The listing builds one solid part. Answer for the finished solid, in the listing's coordinates (mm). A direction names the side the tool comes from. Coordinates: 2 decimals unless noted, no trailing zeros. Order: outer loops, then holes, each group sorted by start corner. A loop starts at its lowest first (then second) coordinate and runs counter-clockwise, first axis right, second up.
from build123d import *

# Parameters (mm, degrees)
BOSS_EXTRUDE1_DEPTH = 30
SKETCH2_W           = 45.814700403
SKETCH2_H           = 10
CUT_EXTRUDE1_DEPTH  = 80
CUT_EXTRUDE2_DEPTH  = 10


with BuildPart() as part:
    # Sketch1 → Boss-Extrude1 (new body)
    with BuildSketch(Plane.XY.offset(3001.335718486)):
        with BuildLine():
            Line((917.934929034, 337.734430273), (888.537204265, 331.753311783))
            ThreePointArc((888.537204265, 331.753311783), (884.042481487, 330.053316774), (880.315998683, 327.019203759))
            Line((880.315998683, 327.019203759), (659.406795905, 282.074088861))
            ThreePointArc((659.406795905, 282.074088861), (654.791020678, 283.41092652), (649.989366626, 283.21952579))
            Line((649.989366626, 283.21952579), (620.591641856, 277.2384073))
            ThreePointArc((620.591641856, 277.2384073), (608.883338717, 259.54898567), (626.572760347, 247.840682531))
            Line((626.572760347, 247.840682531), (655.970485116, 253.821801021))
            ThreePointArc((655.970485116, 253.821801021), (660.465207894, 255.521796031), (664.191690698, 258.555909045))
            Line((664.191690698, 258.555909045), (885.100893475, 303.501023943))
            ThreePointArc((885.100893475, 303.501023943), (889.716668703, 302.164186284), (894.518322755, 302.355587014))
            Line((894.518322755, 302.355587014), (923.916047524, 308.336705504))
            ThreePointArc((923.916047524, 308.336705504), (935.624350664, 326.026127134), (917.934929034, 337.734430273))
        make_face()
        with BuildLine():
            ThreePointArc((618.682580307, 261.542691833), (624.579054184, 257.63992412), (628.481821897, 263.536397997))
            ThreePointArc((628.481821897, 263.536397997), (622.58534802, 267.43916571), (618.682580307, 261.542691833))
        make_face(mode=Mode.SUBTRACT)
        with BuildLine():
            ThreePointArc((916.025867484, 322.038714807), (921.922341361, 318.135947094), (925.825109074, 324.032420971))
            ThreePointArc((925.825109074, 324.032420971), (919.928635197, 327.935188684), (916.025867484, 322.038714807))
        make_face(mode=Mode.SUBTRACT)
    extrude(amount=-BOSS_EXTRUDE1_DEPTH)

    # Sketch2 → Cut-Extrude1 (cut)
    with BuildSketch(Plane(origin=(-23.514742418, 115.577032406, 0), x_dir=(0.9799241589705207, 0.19937061635536468, 0), z_dir=(0.19937061635536468, -0.9799241589705207, 0))):
        with Locations((963.863089214, 2986.335718486)):
            Rectangle(SKETCH2_W, SKETCH2_H)
        with Locations((666.383780489, 2986.335718486)):
            Rectangle(SKETCH2_W, SKETCH2_H)
    extrude(amount=-CUT_EXTRUDE1_DEPTH, mode=Mode.SUBTRACT)

    # Sketch3 → Cut-Extrude2 (cut)
    with BuildSketch(Plane(origin=(-24.112854267, 118.516804882, 0), x_dir=(0.9799241589705208, 0.19937061635536377, 0), z_dir=(0.19937061635536377, -0.9799241589705208, 0))):
        with BuildLine():
            Line((722.337924675, 2993.335718486), (903.120015469, 2993.335718486))
            ThreePointArc((903.120015469, 2993.335718486), (910.120015469, 2986.335718486), (903.120015469, 2979.335718486))
            Line((903.120015469, 2979.335718486), (722.337924675, 2979.335718486))
            ThreePointArc((722.337924675, 2979.335718486), (715.337924675, 2986.335718486), (722.337924675, 2993.335718486))
        make_face()
    cut_extrude2 = extrude(amount=-CUT_EXTRUDE2_DEPTH, mode=Mode.SUBTRACT)

    # Mirror1: Cut-Extrude2 across plane
    add(cut_extrude2.mirror(Plane(origin=(-26.505301663, 130.27589479, 0), x_dir=(0, 0, 1), z_dir=(0.1993706163553639, -0.9799241589705208, 0))), mode=Mode.SUBTRACT)


solid = part.part
1) Each of these flat-tipped pins is pushed along its axis until it touches: P1, Ø5, axis at x = 746.5, z = 2991.5, coming from the -Y side; P2, Ø13, axis at x = 623.58, y = 262.54, coming from the +Z side; P3, Ø6, axis at y = 272.5, z = 2995, coming from the -X side; P4, Ø3, axis at x = 885, z = 2990, coming from the +Y side. Where does it stop, or does it pass through?
2) Section B-B (x = 834) is taken. Give the vertices of the cut face in (y, z).
3) Determine the mould class of faces 1 (the face through (628.49, 261.58, 2976.41)), 2 (the face through (648.99, 267.49, 2986.27)), 3 (the face through (629, 263, 2981.336)), 4 (the face through (915.987, 322.255, 2976.406)) for opening direction X: released by +X, released by -X, zero draft, split by the parting line, or undercut.
4) A tool of negligible diameter and unlimited length cuts with its end or side. For faces 5 (the face through (866.75, 304.8, 2986.49)), 6 (the face through (770, 299, 2979.336)), 7 (the face through (903.442, 334.786, 2993.212)), from which of +Z, -Z, +X, -X, +Y, -Y can it reach the whole face along a straight path? Write none if from no direction.
5) Section D-D (x = 667.5) is taken. Give the vertices of the cut face in (y, z), then the cut area to 3 significant figures.
6) Section A-A (x = 907) is taken. Give the vertices of the cut face in (y, z).
7) Section C-C (z = 2987) is taken. Give the vertices of the cut face in (x, y).
8) Consider L1, parallel to Y at x = 742, z = 2994.5; L2, parallel to Y at x = 689.5, z = 2989; L3, parallel to Y at x = 628, z = 2979.5. Determine where each line is inside the solid, lowest interval first.
Filled sheet:
1. P1: stops at y = 274.96
1. P2: stops at z = 3001.34
1. P3: stops at x = 610.29
1. P4: stops at y = 331.19
2. outline: (293.1, 2971.34) - (317.6, 2971.34) - (317.6, 2979.34) - (307.39, 2979.34) - (307.39, 2993.34) - (317.6, 2993.34) - (317.6, 3001.34) - (293.1, 3001.34) - (293.1, 2993.34) - (303.31, 2993.34) - (303.31, 2979.34) - (293.1, 2979.34) - close
3. face 1: undercut
3. face 2: released by -X
3. face 3: zero draft
3. face 4: undercut
4. face 5: -Y
4. face 6: +Y
4. face 7: +Z, -Z, -X, +Y
5. outline: (259.23, 2971.34) - (283.72, 2971.34) - (283.72, 3001.34) - (259.23, 3001.34) - close
5. area: 735 mm2
6. outline: (304.9, 2971.34) - (335.51, 2971.34) - (335.51, 2981.34) - (304.9, 2981.34) - close; (304.9, 2991.34) - (335.51, 2991.34) - (335.51, 3001.34) - (304.9, 3001.34) - close
7. outline: (645.96, 282.4) - (651.94, 253) - (655.97, 253.82) arc R15 ccw to (664.19, 258.56) - (676.9, 261.14) - (674.9, 270.94) - (865.71, 309.76) - (867.7, 299.96) - (885.1, 303.5) arc R15 ccw to (894.52, 302.36) - (898.55, 303.18) - (892.57, 332.57) - (888.54, 331.75) arc R15 ccw to (880.32, 327.02) - (862.92, 323.48) - (864.91, 313.68) - (674.1, 274.86) - (672.11, 284.66) - (659.41, 282.07) arc R15 ccw to (649.99, 283.22) - close
8. L1: y = 274.39 to 298.88
8. L2: y = 273.91 to 277.99
8. L3: y = 248.13 to 260.2, 264.88 to 278.75
